from build123d import *

# Parameters (mm, degrees)
BASE_PLATE_SKETCH_W        = 180
BASE_PLATE_SKETCH_H        = 90
BASE_PLATE_180X90X22_DEPTH = 22
INCLINED_BOSS_BLOCK_REACH  = 118.629
PIVOT_BOSS_SKETCH_R        = 17.5
PIVOT_BOSS_SKETCH_R_2      = 7.5
PIVOT_BOSS_DEPTH           = 10
CROSS_SLOT_SKETCH_W        = 23
CROSS_SLOT_SKETCH_H        = 90
CROSS_SLOT_23X6_DEPTH      = 6
UPRIGHT_ARM_SKETCH_W       = 90
UPRIGHT_ARM_SKETCH_H       = 125
INCLINED_UPRIGHT_ARM_DEPTH = 22
TOP_PAD_DEPTH              = 20
C_BORE_HOLE_22_D           = 22
C_BORE_HOLE_22_DEPTH       = 22.19797288
C_BORE_HOLE_22_CBORE_D     = 45
C_BORE_HOLE_22_CBORE_DEPTH = 12
TOP_PAD_NOTCHES_DEPTH      = 245.0397404
CROSS_RECESS_SKETCH_W      = 32.386085046
CROSS_RECESS_SKETCH_H      = 28
CROSS_RECESS_SKETCH_W_2    = 30
CROSS_RECESS_5_DEEP_DEPTH  = 5


with BuildPart() as part:
    # Base Plate Sketch → Base Plate 180x90x22 (new body)
    with BuildSketch(Plane(origin=(0, 0, 0), x_dir=(1, 0, 0), z_dir=(0, 1, 0))):
        Rectangle(BASE_PLATE_SKETCH_W, BASE_PLATE_SKETCH_H)
    extrude(amount=BASE_PLATE_180X90X22_DEPTH)

    # Inclined Boss Block Sketch → Inclined Boss Block (add, up to next)
    with BuildSketch(Plane(origin=(0, 35.91019407, 19.905345612), x_dir=(-1, 0, 0), z_dir=(0, -0.874619707139395, -0.48480962024633867)), mode=Mode.PRIVATE) as inclined_boss_block_sk1:
        with BuildLine():
            Line((-4, 11.307924824), (-4, -28.692075176))
            Line((-4, -28.692075176), (-60, -28.692075176))
            Line((-60, -28.692075176), (-60, 11.307924824))
            ThreePointArc((-60, 11.307924824), (-32, 39.307924824), (-4, 11.307924824))
        make_face()
    inclined_boss_block_tool1 = extrude(inclined_boss_block_sk1.sketch, amount=INCLINED_BOSS_BLOCK_REACH, mode=Mode.PRIVATE) - part.part
    add(inclined_boss_block_tool1.solids().sort_by_distance((32, 37.179674, 17.615143))[0])

    # Pivot Boss Sketch → Pivot Boss (add)
    with BuildSketch(Plane(origin=(0, 35.91019407, 19.905345612), x_dir=(1, 0, 0), z_dir=(0, 0.8746197071393949, 0.4848096202463387))):
        with Locations(Location((32, 11.307924824, 0), (0, 0, 90))):
            Circle(PIVOT_BOSS_SKETCH_R)
        with Locations(Location((32, 11.307924824, 0), (0, 0, 270))):
            Circle(PIVOT_BOSS_SKETCH_R_2, mode=Mode.SUBTRACT)
    extrude(amount=PIVOT_BOSS_DEPTH)

    # Cross Slot Sketch → Cross Slot 23x6 (cut)
    with BuildSketch(Plane(origin=(0, 22, 0), x_dir=(1, 0, 0), z_dir=(0, 1, 0))):
        with Locations((-36.5, 0)):
            Rectangle(CROSS_SLOT_SKETCH_W, CROSS_SLOT_SKETCH_H)
    extrude(amount=-CROSS_SLOT_23X6_DEPTH, mode=Mode.SUBTRACT)

    # Upright Arm Sketch → Inclined Upright Arm (add)
    with BuildSketch(Plane(origin=(-60.39090645, -42.286167935, 0), x_dir=(0, 0, -1), z_dir=(0.8191520442889931, 0.5735764363510442, 0))):
        with Locations((0, 114.121879272)):
            Rectangle(UPRIGHT_ARM_SKETCH_W, UPRIGHT_ARM_SKETCH_H)
    extrude(amount=INCLINED_UPRIGHT_ARM_DEPTH)

    # Top Pad Sketch → Top Pad (add)
    with BuildSketch(Plane(origin=(-101.306148094, 144.680173471, 0), x_dir=(0.8191520442889931, 0.5735764363510442, 0), z_dir=(-0.5735764363510442, 0.8191520442889931, 0))):
        with BuildLine():
            Line((-18.723683986, 45), (-73.723683986, 45))
            Line((-73.723683986, 45), (-73.723683986, -45))
            Line((-73.723683986, -45), (-18.723683986, -45))
            ThreePointArc((-18.723683986, -45), (26.276316014, 0), (-18.723683986, 45))
        make_face()
    extrude(amount=-TOP_PAD_DEPTH)

    # C-Bore Hole Ø22
    with Locations(Plane(origin=(-101.306148094, 144.680173471, 0), x_dir=(0.8191520442889931, 0.5735764363510442, 0), z_dir=(-0.5735764363510442, 0.8191520442889931, 0))):
        with Locations((-18.723683986, 0)):
            CounterBoreHole(C_BORE_HOLE_22_D / 2, C_BORE_HOLE_22_CBORE_D / 2, C_BORE_HOLE_22_CBORE_DEPTH, depth=C_BORE_HOLE_22_DEPTH)

    # Top Pad Notch Sketch → Top Pad Notches (cut, through all)
    with BuildSketch(Plane(origin=(-101.306148094, 144.680173471, 0), x_dir=(0.8191520442889931, 0.5735764363510442, 0), z_dir=(-0.5735764363510442, 0.8191520442889931, 0))):
        Polygon((-73.723683986, 20), (-68.723683986, 17.113248654), (-68.723683986, -17.113248654), (-73.723683986, -20), align=None)
    extrude(amount=-TOP_PAD_NOTCHES_DEPTH, mode=Mode.SUBTRACT)

    # Cross Recess Sketch → Cross Recess 5 Deep (cut)
    with BuildSketch(Plane(origin=(-101.306148094, 144.680173471, 0), x_dir=(0.8191520442889931, 0.5735764363510442, 0), z_dir=(-0.5735764363510442, 0.8191520442889931, 0))):
        with Locations((-52.530641463, 0)):
            Rectangle(CROSS_RECESS_SKETCH_W, CROSS_RECESS_SKETCH_H)
        with Locations((13.890230968, 0)):
            Rectangle(CROSS_RECESS_SKETCH_W_2, CROSS_RECESS_SKETCH_H)
    extrude(amount=-CROSS_RECESS_5_DEEP_DEPTH, mode=Mode.SUBTRACT)


solid = part.part
Work out the finished part from the listing and answer in its coordinate system (mm). A direction names the side the tool comes from. Give positions to 0.01 mm unless a question says otherwise; leave off trailing zeros. Write each loop counter-clockwise with the first axis right and the second up, starting at its lowest first coordinate (ties: lowest second). Pieces come first, ordered by that corner, then holes. Notation, with made-up numbers: (11, 31.5) - (35, 31.5) arc R27 ccw to (35, 66.5) - close; hole circle Ø9 at (47, -21). An arc over 180 degrees is marked (long way). One line per item, written item: value. Start each with the question number.
1. Find section A-A (z = 33). Write down the section's boundary in (x, y).
2. Given pin 1 (1.8 mm diameter, centred on y = 17.5, z = 19.5, fed in from -X); pin 2 (3 mm diameter, centred on y = 94, z = 10, fed in from +X); pin 3 (1 mm diameter, centred on y = 16, z = -27, fed in from -X), each flat-ended and moving along its own axis, determine where each tip first touches the part or whether it passes through.
3. For a pull along Z with two mould halves and no side action, classify faces 1 (the flat face through (-51, 21, 45)), 2 (the flat face through (-100.7, 120.69, -10.63)), 3 (the cylindrical face through (24.68, 46.49, 10.98)) as +Z half, -Z half, draft (parallel to the pull), parting line (faces both ways), or undercut.
4. Consider probe 1 along Y at (x, z) = (-32, 14.5); probe 2 along Y at (x, z) = (-79.5, 15); probe 3 along Y at (x, z) = (-82, -25). Determine where each line is inside the solid, lowest interval first.
5. Find section D-D (x = 6.5). Write down the section's boundary in (y, z), then the cut area to 3 significant figures.
6. Find section B-B (x = -32.5). Write down the section's boundary in (y, z).
7. For faces 4 (the flat face through (35.644, 53.791, 8.275)), 5 (the flat face through (-48, 19, 1)), 6 (the flat face through (19, 22, -31)), determine the directions among +Z, -Z, +X, -X, +Y, -Y from which every point of the face is accessible in a straight line to the end or side of a thin tool.
8. Find section C-C (y = 94). Write down the section's boundary in (x, z).
Geometry results:
1. outline: (-161.7, 102.39) - (-90, 0) - (90, 0) - (90, 22) - (60, 22) - (60, 28.65) - (4, 28.65) - (4, 22) - (-25, 22) - (-25, 16) - (-48, 16) - (-48, 22) - (-78.55, 22) - (-132.2, 98.63) - (-80.11, 135.11) - (-91.58, 151.49) - close
2. pin 1: x = -102.78
2. pin 2: x = -127.91
2. pin 3: x = -101.55
3. face 1: +Z half
3. face 2: draft
3. face 3: undercut
4. probe 1: 0 to 16
4. probe 2: 0 to 23.36, 135.53 to 154.86
4. probe 3: 0 to 26.93, 133.78 to 149.7
5. outline: (0, -45) - (22, -45) - (22, -13.96) - (47, -0.1) - (22, 45) - (0, 45) - close
5. area: 2,720 mm2
6. outline: (0, -45) - (16, -45) - (16, 45) - (0, 45) - close
7. face 4: +Z, +X, +Y
7. face 5: +Z, -Z, +Y
7. face 6: -Z, +Y
8. outline: (-155.82, -45) - (-128.96, -45) - (-128.96, 45) - (-155.82, 45) - (-155.82, 20) - (-149.72, 17.11) - (-149.72, -17.11) - (-155.82, -20) - close
